from build123d import *

# Parameters (mm, degrees)
BASE_PLATE_SKETCH_R  = 7.5
BASE_PLATE_DEPTH     = 15
UPRIGHT_WEB_SKETCH_R = 7.5
UPRIGHT_WEB_DEPTH    = 15
COLUMN_DEPTH         = 15
SWIVEL_START         = -50
SWIVEL_HEAD_SKETCH_R = 7.5
SWIVEL_HEAD_DEPTH    = 50
GUSSET_SKETCH_R      = 7.5
GUSSET_DEPTH         = 10
PIVOT_START          = -40
PIVOT_HOLE_SKETCH_R  = 7.5
PIVOT_HOLE_DEPTH     = 40


with BuildPart() as part:
    # Base Plate Sketch → Base Plate (new body)
    with BuildSketch(Plane(origin=(0, 0, 0), x_dir=(1, 0, 0), z_dir=(0, 1, 0))):
        with BuildLine():
            Line((17.13196958, 75.51487018), (-12.86803042, 5.51487018))
            ThreePointArc((-12.86803042, 5.51487018), (-11.687775291, -7.706874122), (0, -14))
            Line((0, -14), (60, -14))
            ThreePointArc((60, -14), (71.687775291, -7.706874122), (72.86803042, 5.51487018))
            Line((72.86803042, 5.51487018), (42.86803042, 75.51487018))
            ThreePointArc((42.86803042, 75.51487018), (30, 84), (17.13196958, 75.51487018))
        make_face()
        with Locations(Location((0, 0, 0), (0, 0, 270))):
            Circle(BASE_PLATE_SKETCH_R, mode=Mode.SUBTRACT)
        with Locations(Location((60, 0, 0), (0, 0, 270))):
            Circle(BASE_PLATE_SKETCH_R, mode=Mode.SUBTRACT)
        with Locations(Location((30, 70, 0), (0, 0, 270))):
            Circle(BASE_PLATE_SKETCH_R, mode=Mode.SUBTRACT)
    extrude(amount=BASE_PLATE_DEPTH)

    # Upright Web Sketch → Upright Web (add)
    with BuildSketch(Plane.XZ):
        with BuildLine():
            Line((-12.86803042, -5.51487018), (11.049826186, -76.394600254))
            ThreePointArc((11.049826186, -76.394600254), (30, -90), (48.950173814, -76.394600254))
            Line((48.950173814, -76.394600254), (72.86803042, -5.51487018))
            ThreePointArc((72.86803042, -5.51487018), (71.687775291, 7.706874122), (60, 14))
            Line((60, 14), (44, 14))
            ThreePointArc((44, 14), (30, 28), (16, 14))
            Line((16, 14), (0, 14))
            ThreePointArc((0, 14), (-11.687775291, 7.706874122), (-12.86803042, -5.51487018))
        make_face()
        with Locations((30, 14)):
            Circle(UPRIGHT_WEB_SKETCH_R, mode=Mode.SUBTRACT)
        with Locations(Location((0, 0, 0), (0, 0, 90))):
            Circle(UPRIGHT_WEB_SKETCH_R, mode=Mode.SUBTRACT)
        with Locations(Location((60, 0, 0), (0, 0, 90))):
            Circle(UPRIGHT_WEB_SKETCH_R, mode=Mode.SUBTRACT)
    extrude(amount=-UPRIGHT_WEB_DEPTH)

    # Column Sketch → Column (add)
    with BuildSketch(Plane(origin=(0, 15, 0), x_dir=(1, 0, 0), z_dir=(0, 1, 0))):
        with BuildLine():
            ThreePointArc((11.049826186, 76.394600254), (10.264201609, 73.240102137), (10, 70))
            Line((10, 70), (10.203045685, 67.157360406))
            Line((10.203045685, 67.157360406), (16, -14))
            ThreePointArc((16, -14), (30, -28), (44, -14))
            Line((44, -14), (49.796954315, 67.157360406))
            Line((49.796954315, 67.157360406), (50, 70))
            ThreePointArc((50, 70), (49.735798391, 73.240102137), (48.950173814, 76.394600254))
            ThreePointArc((48.950173814, 76.394600254), (30, 90), (11.049826186, 76.394600254))
        make_face()
        with BuildLine():
            ThreePointArc((37.5, -14), (30, -21.5), (22.5, -14))
            ThreePointArc((22.5, -14), (30, -6.5), (37.5, -14))
        make_face(mode=Mode.SUBTRACT)
    extrude(amount=COLUMN_DEPTH)

    # Swivel Head Sketch → Swivel Head (add)
    with BuildSketch(Plane(origin=(0, 72, 0), x_dir=(1, 0, 0), z_dir=(0, 1, 0)).offset(SWIVEL_START)):
        with BuildLine():
            ThreePointArc((17.018262435, 54.785714286), (30, 56), (42.981737565, 54.785714286))
            Line((42.981737565, 54.785714286), (49.550987537, 63.713825524))
            Line((49.550987537, 63.713825524), (49.796954315, 67.157360406))
            Line((49.796954315, 67.157360406), (50, 70))
            ThreePointArc((50, 70), (30, 90), (10, 70))
            Line((10, 70), (10.203045685, 67.157360406))
            Line((10.203045685, 67.157360406), (10.449012463, 63.713825524))
            Line((10.449012463, 63.713825524), (17.018262435, 54.785714286))
        make_face()
        with Locations(Location((30, 70, 0), (0, 0, 270))):
            Circle(SWIVEL_HEAD_SKETCH_R, mode=Mode.SUBTRACT)
    extrude(amount=SWIVEL_HEAD_DEPTH)

    # Gusset Sketch → Gusset (add)
    with BuildSketch(Plane(origin=(0, 72, 0), x_dir=(1, 0, 0), z_dir=(0, 1, 0))):
        with BuildLine():
            ThreePointArc((58.635369301, 49.875), (30, 105), (1.364630699, 49.875))
            ThreePointArc((1.364630699, 49.875), (30, 56), (58.635369301, 49.875))
        make_face()
        with Locations(Location((30, 70, 0), (0, 0, 270))):
            Circle(GUSSET_SKETCH_R, mode=Mode.SUBTRACT)
    extrude(amount=GUSSET_DEPTH)

    # Pivot Hole Sketch → Pivot Hole (cut)
    with BuildSketch(Plane(origin=(0, 30, 0), x_dir=(1, 0, 0), z_dir=(0, 1, 0)).offset(PIVOT_START)):
        with Locations(Location((30, 70, 0), (0, 0, 270))):
            Circle(PIVOT_HOLE_SKETCH_R)
    extrude(amount=PIVOT_HOLE_DEPTH, mode=Mode.SUBTRACT)


solid = part.part
Build history of the part. All positions in model axes, mm. A direction names the side the tool comes from. Round coordinates to 2 decimals unless told otherwise and drop trailing zeros. Write each loop counter-clockwise with the first axis right and the second up, starting at its lowest first coordinate (ties: lowest second). Pieces come first, ordered by that corner, then holes. Notation, with made-up numbers: (0.25, 28.5) -> (9.25, 28.5) arc R17 ccw to (9.25, 53.5) -> close; hole circle Ø3 at (2, 83). An arc over 180 degrees is marked (long way). Use one line per item in the form item = value.
Q1. Drop flat-ended pins along their axis: P1, Ø9, axis at x = 30, z = 14, coming from the +Y side; P2, Ø7.5, axis at x = 5.5, y = 4, coming from the +Z side; P3, Ø11.5, axis at x = 30.5, z = 1.5, coming from the +Y side; P4, Ø9, axis at x = 0, z = 0, coming from the +Y side. Give the stop position or say it passes through.
Conclusion:
P1 = 15
P2 = 14
P3 = 30
P4 = through
Q2. Band-saw the part on D-D, the plane z = 19. Write the cut outline in (x, y).
Conclusion:
outline = (16.92, 0) -> (24.41, 0) -> (24.41, 30) -> (16.92, 30) -> close; (35.59, 0) -> (43.08, 0) -> (43.08, 30) -> (35.59, 30) -> close
Q3. Two-plate mould, pull along X, no slides. Class faces 1 (the flat face through (30, 15, 11)), 2 (the flat face through (8, 7, 14)), 3 (the flat face through (30, 7, 14)), 4 (the cylindrical face through (30, 15, 28)): released by +X, released by -X, zero draft, split by the parting line, or undercut.
Conclusion:
face_1 = undercut
face_2 = zero draft
face_3 = undercut
face_4 = split by the parting line
Q4. Tool access for faces 5 (the flat face through (52, 7, 14)), 6 (the flat face through (60.74, 7.4, -41.45)), 7 (the cylindrical face through (31.63, 18.12, 21.32)), 8 (the flat face through (46.22, 50.71, -59.19)), 9 (the flat face through (-1.077, 7.395, -40.459)): list every direction of +Z, -Z, +X, -X, +Y, -Y with a clear straight run to the whole face (end or side of a thin tool).
Conclusion:
face_5 = +Z, +X, +Y, -Y
face_6 = -Z, +X, -Y
face_7 = +Y
face_8 = +Z, +X
face_9 = -Z, -X, -Y
Q5. Band-saw the part on A-A, the plane z = 0. Write the cut outline in (x, y).
Conclusion:
outline = (-14, 0) -> (-7.5, 0) -> (-7.5, 15) -> (-14, 15) -> close; (7.5, 0) -> (52.5, 0) -> (52.5, 15) -> (45, 15) -> (45, 30) -> (15, 30) -> (15, 15) -> (7.5, 15) -> close; (67.5, 0) -> (74, 0) -> (74, 15) -> (67.5, 15) -> close
Q6. Band-saw the part on C-C, the plane y = 35. Write the cut outline in (x, z), then the cut area to 3 significant figures.
Conclusion:
outline = (10, -70) arc R20 ccw to (50, -70) -> (49.55, -63.71) -> (42.98, -54.79) arc R70 cw to (17.02, -54.79) -> (10.45, -63.71) -> close; hole circle Ø15 at (30, -70)
area = 970 mm²
Q7. Drill centre lines: L1, parallel to X at y = 3.75, z = 0; L2, parallel to Z at x = 30, y = 19.5; L3, parallel to X at y = 61.5, z = -70. Where is each one in solid material? Low to high.
Conclusion:
L1 = -14 to -7.5, 7.5 to 52.5, 67.5 to 74
L2 = -90 to -77.5, -62.5 to 6.5, 21.5 to 28
L3 = 10 to 22.5, 37.5 to 50
Q8. Band-saw the part on B-B, the plane x = 30. Write the cut outline in (y, z).
Conclusion:
outline = (0, -90) -> (72, -90) -> (72, -105) -> (82, -105) -> (82, -77.5) -> (0, -77.5) -> close; (0, -62.5) -> (82, -62.5) -> (82, -56) -> (30, -56) -> (30, 6.5) -> (15, 6.5) -> (15, 14) -> (0, 14) -> close; (0, 21.5) -> (30, 21.5) -> (30, 28) -> (0, 28) -> close
